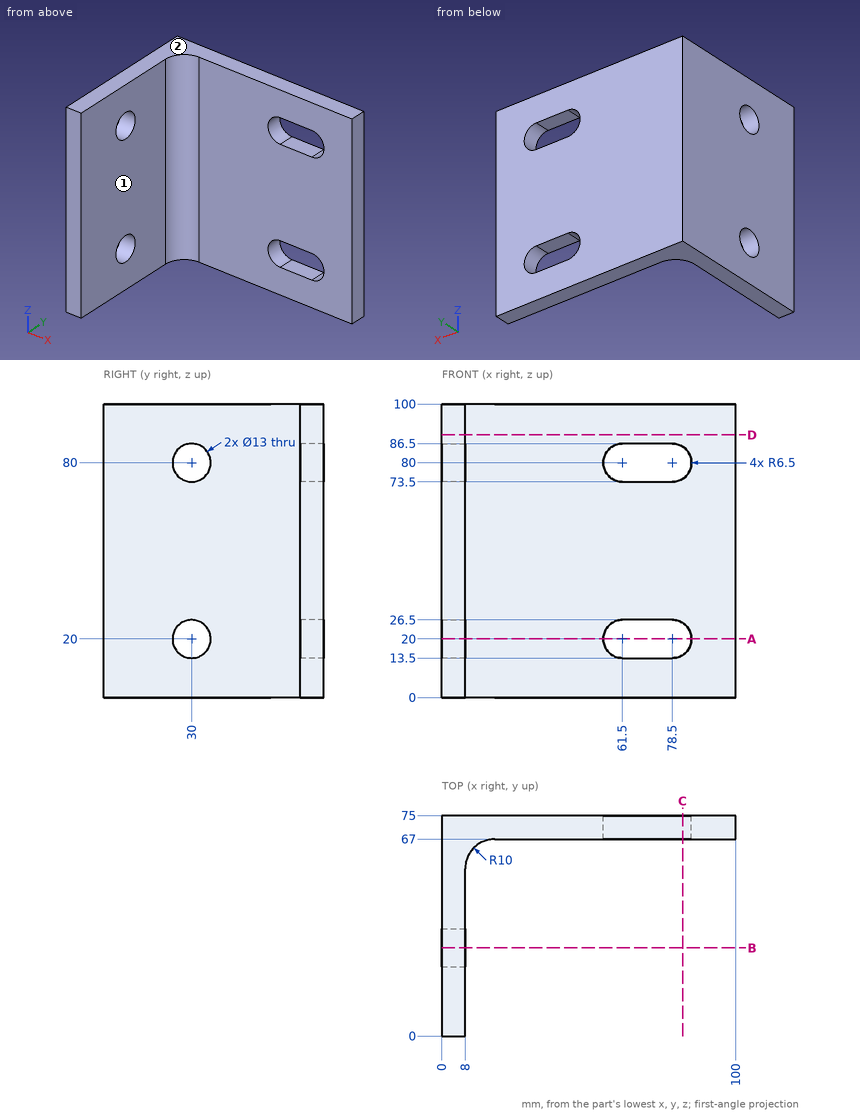
Input: dimensioned drawing with shaded views. Units: mm. Origin: part minimum x, y, z. A direction names the side the tool comes from. Round coordinates to 2 decimals unless told otherwise and drop trailing zeros. Loops run counter-clockwise (first coordinate to the right, second up) from the corner with the lowest first, then second, coordinate; pieces in that order, holes last. Notation, with made-up numbers: (64, -20) -> (113, -20) arc R13 ccw to (113, 0) -> close; hole circle Ø5 at (81.5, -23). An arc over 180 degrees is marked (long way). Answer as a JSON object with one key per item and string values. Group by question number.
1) Section query B-B on y = 30. Output: boundary loops of the cut face in (x, z), plus the area to 3 significant figures.
2) Section query A-A on z = 20. Output: boundary loops of the cut face in (x, y), plus the area to 3 significant figures.
3) Section query C-C on x = 82. Output: boundary loops of the cut face in (y, z), plus the area to 3 significant figures.
4) Pin query (flat end, axial travel): pin 1 (3 mm diameter, centred on x = 61, z = 40, fed in from -Y); pin 2 (21 mm diameter, centred on y = 30, z = 20, fed in from -X); pin 3 (1 mm diameter, centred on y = 49, z = 10.5, fed in from +X); pin 4 (11.5 mm diameter, centred on y = 30, z = 80, fed in from +X). Return the tip coordinate at first contact, or that it passes through.
5) Section query D-D on z = 89.5. Output: boundary loops of the cut face in (x, y).
6) Ray query, L1, parallel to Y at x = 6, z = 20; L2, parallel to Y at x = 83, z = 57; L3, parallel to X at y = 18.5, z = 59. Return the intervals inside material, ascending.
7) Reachability of the marked faces 1 and 2 from +Z, -Z, +X, -X, +Y, -Y: full face, straight path, thin tool, end or side. Return the list, or none.
Reply:
{
 "1": {"outline": "(0, 0) -> (8, 0) -> (8, 13.5) -> (0, 13.5) -> close; (0, 26.5) -> (8, 26.5) -> (8, 73.5) -> (0, 73.5) -> close; (0, 86.5) -> (8, 86.5) -> (8, 100) -> (0, 100) -> close", "area": "592 mm2"},
 "2": {"outline": "(0, 0) -> (8, 0) -> (8, 23.5) -> (0, 23.5) -> close; (0, 36.5) -> (8, 36.5) -> (8, 57) arc R10 cw to (18, 67) -> (55, 67) -> (55, 75) -> (0, 75) -> close; (85, 67) -> (100, 67) -> (100, 75) -> (85, 75) -> close", "area": "1,010 mm2"},
 "3": {"outline": "(67, 0) -> (75, 0) -> (75, 14.52) -> (67, 14.52) -> close; (67, 25.48) -> (75, 25.48) -> (75, 74.52) -> (67, 74.52) -> close; (67, 85.48) -> (75, 85.48) -> (75, 100) -> (67, 100) -> close", "area": "625 mm2"},
 "4": {"pin 1": "stops at y = 67", "pin 2": "stops at x = 0", "pin 3": "stops at x = 8", "pin 4": "passes through"},
 "5": {"outline": "(0, 0) -> (8, 0) -> (8, 57) arc R10 cw to (18, 67) -> (100, 67) -> (100, 75) -> (0, 75) -> close"},
 "6": {"L1": "y = 0 to 23.5, 36.5 to 75", "L2": "y = 67 to 75", "L3": "x = 0 to 8"},
 "7": {"face 1": "+Z, -Z, +X, -Y", "face 2": "+Z, +X, -X, +Y, -Y"}
}
